Could you check a few things on this model? Use its own coordinates, in mm. Face numbers are marked on the shaded views. A direction names the side the tool comes from. Round coordinates to 2 decimals unless told otherwise and drop trailing zeros. Order: outer loops, then holes, each group sorted by start corner. A loop starts at its lowest first (then second) coordinate and runs counter-clockwise, first axis right, second up.
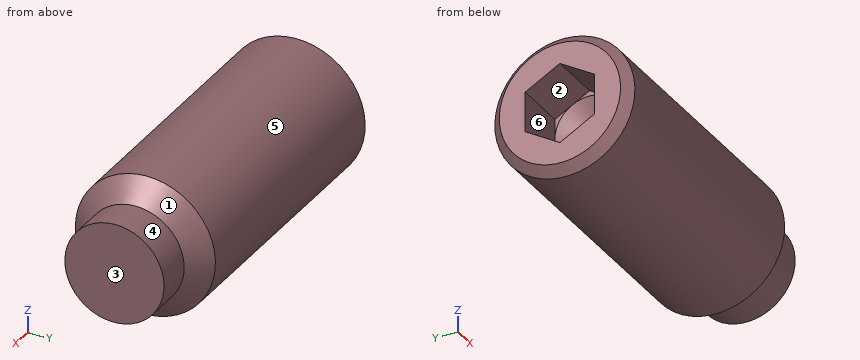
```python
from build123d import *

# Parameters (mm, degrees)
CUT_EXTRUDE_1_DEPTH = 4.8


with BuildPart() as part:
    # 草图1 → Revolve 598 (revolve)
    with BuildSketch(Plane.XY, mode=Mode.PRIVATE) as revolve_598_sk:
        Polygon((0, 0), (30, 0), (30, 4.25), (26.75, 4.25), (25, 6), (0.804, 6), (0, 5.196), align=None)
    revolve(revolve_598_sk.sketch.rotate(Axis((-0.665465891, 0, 0), (1, 0, 0)), 90), axis=Axis((-0.665465891, 0, 0), (1, 0, 0)))

    # 草图2 → 切除-拉伸1 (cut)
    with BuildSketch(Plane.ZY):
        Polygon((3.43, 0), (1.715, 2.970467135), (-1.715, 2.970467135), (-3.43, 0), (-1.715, -2.970467135), (1.715, -2.970467135), align=None)
    extrude(amount=-CUT_EXTRUDE_1_DEPTH, mode=Mode.SUBTRACT)

    # 草图3 → 切除-旋转1 (revolve, cut)
    with BuildSketch(Plane.XY, mode=Mode.PRIVATE) as cut_revolve_1_sk:
        Polygon((4.8, 2.970467135), (6.515, 0), (4.8, 0), align=None)
    revolve(cut_revolve_1_sk.sketch.rotate(Axis((-0.262128326, 0, 0), (1, 0, 0)), 90), axis=Axis((-0.262128326, 0, 0), (1, 0, 0)), mode=Mode.SUBTRACT)


solid = part.part
```
Q1. For the marked faces 4, 5 and 6, which set-ups out of +Z, -Z, +X, -X, +Y, -Y let a thin tool reach every point of the face, with its end or its side?
Q2. I need wall thicknesses on L1, parallel to Z at x = 2.5, y = -1.5; L2, parallel to Z at x = 24.5, y = -3; L3, parallel to X at y = -2, z = 0.5. Which ranges of each line are inside material? Lowest first, please.
Q3. For P1, Ø3, axis at x = 15, y = -4, coming from the -Z side; P2, Ø4, axis at x = 3, z = 0.5, coming from the +Y side; P3, Ø4, axis at x = 21.5, z = 4, coming from the -Y side; P4, Ø3, axis at x = 10, y = 2, coming from the +Z side, each with a flat end and sliding along its axis, tell me the tip position at first contact or that it passes through.
Q4. We'd pull the mould along Y, two halves only. Please class the marked faces 1, 2 and 3: released by +Y, released by -Y, zero draft, split by the parting line, or undercut.
Q5. Imagine slicing it at A-A, the plane x = 21.25. Please give me the cut outline in (y, z), then the cut area to 3 significant figures.
Filled in:
1. face 4: +X
1. face 5: +X, -X
1. face 6: -X
2. L1: z = -5.81 to -2.56, 2.56 to 5.81
2. L2: z = -5.2 to 5.2
2. L3: x = 5.32 to 30
3. P1: stops at z = -5.45
3. P2: stops at y = 6
3. P3: stops at y = -5.66
3. P4: stops at z = 5.98
4. face 1: split by the parting line
4. face 2: undercut
4. face 3: zero draft
5. outline: circle Ø12 at (0, 0)
5. area: 113 mm2
